```python
from build123d import *

# Parameters (mm, degrees)
BASE_EXTRUDE_DEPTH = 7.5
SKETCH4_W          = 0.6
SKETCH4_H          = 11.392304845
CHAMFER_2_SIZE     = 1.4
FILLET_2_R         = 0.6


with BuildPart() as part:
    # Sketch1 → Base-extrude (new body)
    with BuildSketch(Plane(origin=(0, 0, 0), x_dir=(0, 0, -1), z_dir=(1, 0, 0))):
        Polygon((9, 5.196152423), (9, -5.196152423), (0, -10.392304845), (-9, -5.196152423), (-9, 5.196152423), (0, 10.392304845), align=None)
    extrude(amount=BASE_EXTRUDE_DEPTH)

    # Sketch2 → Boss-Revolve1 (revolve)
    with BuildSketch(Plane.XY, mode=Mode.PRIVATE) as boss_revolve1_sk:
        Polygon((0, 0), (107.5, 0), (107.5, 4.4845), (107.5, 6), (7.791693541, 6), (0, 6), align=None)
    revolve(boss_revolve1_sk.sketch.rotate(Axis((0, 0, 0), (1, 0, 0)), 90), axis=Axis((0, 0, 0), (1, 0, 0)))

    # Sketch3 → Cut-Revolve1 (revolve, cut)
    with BuildSketch(Plane.XY):
        Polygon((0, 9), (3.690598923, 15.392304845), (3.690598923, 20.392304845), (-10, 20.392304845), (-10, 9), align=None)
    revolve(axis=Axis((0, 0, 0), (1, 0, 0)), mode=Mode.SUBTRACT)

    # Sketch5 → Cut-Revolve2 (revolve, cut)
    with BuildSketch(Plane.XY):
        Polygon((7.5, 9), (3.809401077, 15.392304845), (3.809401077, 20.392304845), (13.809401077, 20.392304845), (13.809401077, 9), align=None)
    revolve(axis=Axis((0, 0, 0), (1, 0, 0)), mode=Mode.SUBTRACT)

    # Sketch4 → Cut-Revolve3 (revolve, cut)
    with BuildSketch(Plane.XY, mode=Mode.PRIVATE) as cut_revolve3_sk:
        with Locations((7.2, 14.696152423)):
            Rectangle(SKETCH4_W, SKETCH4_H)
    revolve(cut_revolve3_sk.sketch.rotate(Axis((0, 0, 0), (1, 0, 0)), 270), axis=Axis((0, 0, 0), (1, 0, 0)), mode=Mode.SUBTRACT)

    # Chamfer 2
    chamfer_2_edges = [part.edges().sort_by_distance(p)[0] for p in [
        (107.5, 0, -6),
    ]]
    chamfer(chamfer_2_edges, length=CHAMFER_2_SIZE)

    # Fillet 2
    fillet_2_edges = [part.edges().sort_by_distance(p)[0] for p in [
        (7.5, 0, -6),
    ]]
    fillet(fillet_2_edges, radius=FILLET_2_R)


solid = part.part
```
Check sheet for the modelled part. Datum: model origin and axes. Units: mm. A direction names the side the tool comes from. Round coordinates to 2 decimals unless told otherwise and drop trailing zeros. Loops run counter-clockwise (first coordinate to the right, second up) from the corner with the lowest first, then second, coordinate; pieces in that order, holes last. Notation, with made-up numbers: M 57.5,74.25 L 83.5,74.25 A35 ccw 83.5,109.25 Z; hole C 7.25,39 d4. An arc over 180 degrees is marked long. Answer as a JSON object with one key per item and string values.
1. Access from +Z, -Z, +X, -X, +Y, -Y to the whole of each face (thin tool, end or side, straight path). Record for faces 1 (the flat face through (6.9, -5, -8)), 2 (the flat face through (6.9, 4.5, -8.1)), 3 (the cylindrical face through (7.2, -5.48, 7.14)), 4 (the flat face through (6.9, -9.3, 0)).
Reply:
{"face 1": "-Z, +X, -Y", "face 2": "-Z, +X, +Y", "face 3": "+X", "face 4": "+X, -Y"}
2. Gauge pin test, flat ends, axial feed: P1, Ø1.3, axis at y = 3.5, z = -6, coming from the +X side; P2, Ø3, axis at x = 70, z = -6.5, coming from the -Y side; P3, Ø5, axis at x = 23.5, y = -2, coming from the +Z side. Record the tip position at first contact, or that the pin passes through.
Reply:
{"P1": "stops at x = 7.58", "P2": "stops at y = -3.32", "P3": "stops at z = 6"}
3. Section check A-A (x = 85.5). Record the boundary of the cut face in (y, z).
Reply:
{"outline": "C 0,0 d12"}
4. Scan lines: line 1 (Y direction, x = 83, z = 0.5); line 2 (Y direction, x = 22, z = 2.25); line 3 (X direction, y = -2.5, z = 6.25). Record each from-to range of solid material in increasing order.
Reply:
{"line 1": "y = -5.98 to 5.98", "line 2": "y = -5.56 to 5.56", "line 3": "x = 0 to 7.5"}
